```python
from build123d import *

# Parameters (mm, degrees)
SKETCH1_R           = 35
BOSS_EXTRUDE1_DEPTH = 10
CHAMFER1_SIZE       = 1
SKETCH2_R           = 10
CUT_EXTRUDE1_DEPTH  = 30
SKETCH3_R           = 3.5
CUT_EXTRUDE2_DEPTH  = 29


with BuildPart() as part:
    # Sketch1 → Boss-Extrude1 (new body)
    with BuildSketch(Plane.XY):
        Circle(SKETCH1_R)
    extrude(amount=BOSS_EXTRUDE1_DEPTH)

    # Chamfer1
    chamfer1_edges = [part.edges().sort_by_distance(p)[0] for p in [
        (-35, 0, 0),
        (-35, 0, 10),
    ]]
    chamfer(chamfer1_edges, length=CHAMFER1_SIZE)

    # Sketch2 → Cut-Extrude1 (cut)
    with BuildSketch(Plane.XY.offset(10)):
        Circle(SKETCH2_R)
    extrude(amount=-CUT_EXTRUDE1_DEPTH, mode=Mode.SUBTRACT)

    # Sketch3 → Cut-Extrude2 (cut)
    with BuildSketch(Plane.XY.offset(10)):
        with Locations((27.5, 0)):
            Circle(SKETCH3_R)
    extrude(amount=-CUT_EXTRUDE2_DEPTH, mode=Mode.SUBTRACT)


solid = part.part
```
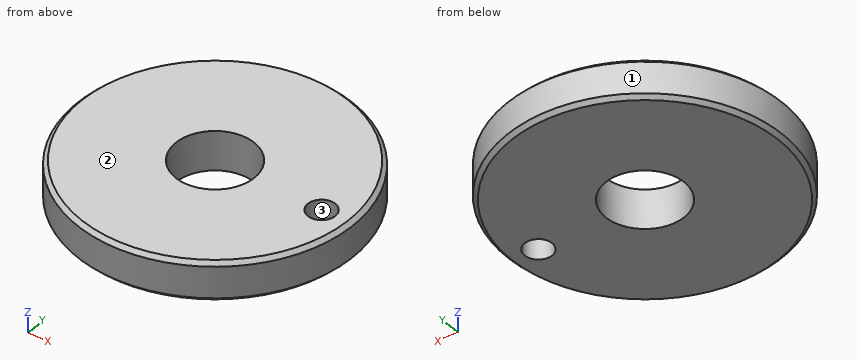
The listing builds one solid part. Answer for the finished solid, in the listing's coordinates (mm). Face numbers are marked on the shaded views. Coordinates: 2 decimals unless noted, no trailing zeros. Write each loop counter-clockwise with the first axis right and the second up, starting at its lowest first coordinate (ties: lowest second). Pieces come first, ordered by that corner, then holes. Notation, with made-up numbers: (-15.75, 87) - (-4.75, 87) arc R29 ccw to (-4.75, 108) - close; hole circle Ø2 at (38, 27.25). An arc over 180 degrees is marked (long way). Return JSON: item names as keys, results as strings. Group by question number.
1. A cutting plane is placed at A-A, the plane x = 0. Determine the outline of the cut face in (y, z), plus the area to 3 significant figures.
2. Given pin 1 (4 mm diameter, centred on x = 26, z = 7, fed in from +Y); pin 2 (1 mm diameter, centred on x = -28, z = 7.5, fed in from -Y); pin 3 (5 mm diameter, centred on y = -9, z = 6.5, fed in from -X); pin 4 (5 mm diameter, centred on x = -10.5, y = 3.5, fed in from -Z), each flat-ended and moving along its own axis, determine where each tip first touches the part or whether it passes through.
3. A cutting plane is placed at C-C, the plane z = 7.75. Determine the outline of the cut face in (x, y), plus the area to 3 significant figures.
4. Determine the mould class of the marked faces 1, 2 and 3 for opening direction X: released by +X, released by -X, zero draft, split by the parting line, or undercut.
5. A cutting plane is placed at B-B, the plane y = 0. Determine the outline of the cut face in (x, z).
6. Straight lines are drawn through the part: L1, parallel to Y at x = 0, z = 3; L2, parallel to Y at x = 5.5, z = 7.25; L3, parallel to X at y = 9, z = 3.5. For each, find the intervals that lie inside material, in ascending order.
Ans:
{
 "1": {"outline": "(-35, 1) - (-34, 0) - (-10, 0) - (-10, 10) - (-34, 10) - (-35, 9) - close; (10, 0) - (34, 0) - (35, 1) - (35, 9) - (34, 10) - (10, 10) - close", "area": "498 mm²"},
 "2": {"pin 1": "y = 25.48", "pin 2": "y = -21.65", "pin 3": "x = -34.39", "pin 4": "z = 0"},
 "3": {"outline": "circle Ø70 at (0, 0); hole circle Ø20 at (0, 0); hole circle Ø7 at (27.5, 0)", "area": "3,500 mm²"},
 "4": {"face 1": "split by the parting line", "face 2": "zero draft", "face 3": "undercut"},
 "5": {"outline": "(-35, 1) - (-34, 0) - (-10, 0) - (-10, 10) - (-34, 10) - (-35, 9) - close; (10, 0) - (24, 0) - (24, 10) - (10, 10) - close; (31, 0) - (34, 0) - (35, 1) - (35, 9) - (34, 10) - (31, 10) - close"},
 "6": {"L1": "-35 to -10, 10 to 35", "L2": "-34.57 to -8.35, 8.35 to 34.57", "L3": "-33.82 to -4.36, 4.36 to 33.82"}
}
